```python
from build123d import *

# Parameters (mm, degrees)
SPANNER_BODY_3MM_DEPTH          = 3
HEAD_PAD_13_SIDE_A_DEPTH        = 1
HEAD_START                      = 1
HEAD_PAD_13_SIDE_B_DEPTH        = 1
HEAD_PAD_9_SIDE_A_DEPTH         = 1
HEAD_PAD_9_SIDE_B_DEPTH         = 1
HANDLE_SLOT_SIDE_A_55X6_5_DEPTH = 0.7
HANDLE_SLOT_SIDE_B_55X6_5_DEPTH = 0.7


with BuildPart() as part:
    # Spanner Profile Sketch → Spanner Body 3mm (new body)
    with BuildSketch(Plane.XY):
        with BuildLine():
            ThreePointArc((0.335793671, 9.351551373), (4.669621374, 5.426922629), (6.845232579, 0))
            Line((6.845232579, 0), (107.225035612, 0))
            ThreePointArc((107.225035612, 0), (107.061451957, 3.049932803), (107.927329677, 5.978943813))
            Line((107.927329677, 5.978943813), (120.095812241, 10.407909262))
            ThreePointArc((120.095812241, 10.407909262), (111.608728128, 14.410482081), (102.447920261, 12.37804878))
            ThreePointArc((102.447920261, 12.37804878), (90.682307093, 7.25217294), (77.968765244, 5.5))
            Line((77.968765244, 5.5), (34.824560299, 5.5))
            ThreePointArc((34.824560299, 5.5), (21.256828973, 7.500925935), (8.844332774, 13.333333333))
            ThreePointArc((8.844332774, 13.333333333), (-5.944434547, 14.854753378), (-15.600963823, 3.551046014))
            Line((-15.600963823, 3.551046014), (0.335793671, 9.351551373))
        make_face()
        with BuildLine():
            Line((107.225035612, 0), (6.845232579, 0))
            ThreePointArc((6.845232579, 0), (6.928993977, -3.356876833), (6.150136107, -6.623223181))
            Line((6.150136107, -6.623223181), (-9.990209349, -12.497828498))
            ThreePointArc((-9.990209349, -12.497828498), (0.615850097, -15.988143377), (10.921993446, -11.692307692))
            ThreePointArc((10.921993446, -11.692307692), (18.183666088, -7.104008283), (26.622359024, -5.5))
            Line((26.622359024, -5.5), (85.627884786, -5.5))
            ThreePointArc((85.627884786, -5.5), (93.595318501, -6.924087505), (100.576115451, -11.02))
            ThreePointArc((100.576115451, -11.02), (115.204003038, -13.533970311), (124.379255248, -1.867356026))
            Line((124.379255248, -1.867356026), (112.37359154, -6.237060258))
            ThreePointArc((112.37359154, -6.237060258), (109.059269326, -3.729420365), (107.225035612, 0))
        make_face()
    extrude(amount=SPANNER_BODY_3MM_DEPTH)

    # Head Pad 13 Side A Sketch → Head Pad 13 Side A (add)
    with BuildSketch(Plane.XY.offset(3)):
        with BuildLine():
            Line((-15.600963823, 3.551046014), (0.335793671, 9.351551373))
            ThreePointArc((0.335793671, 9.351551373), (6.21600407, 2.446261863), (6.150136107, -6.623223181))
            Line((6.150136107, -6.623223181), (-9.990209349, -12.497828498))
            ThreePointArc((-9.990209349, -12.497828498), (15.10359657, 5.280281303), (-15.600963823, 3.551046014))
        make_face()
    extrude(amount=HEAD_PAD_13_SIDE_A_DEPTH)

    # Head Pad 13 Side B Sketch → Head Pad 13 Side B (add)
    with BuildSketch(Plane(origin=(0, 0, 0), x_dir=(-1, 0, 0), z_dir=(0, 0, -1)).offset(HEAD_START)):
        with BuildLine():
            Line((-0.335793671, 9.351551373), (15.600963823, 3.551046014))
            ThreePointArc((15.600963823, 3.551046014), (-15.10359657, 5.280281303), (9.990209349, -12.497828498))
            Line((9.990209349, -12.497828498), (-6.150136107, -6.623223181))
            ThreePointArc((-6.150136107, -6.623223181), (-6.21600407, 2.446261863), (-0.335793671, 9.351551373))
        make_face()
    extrude(amount=-HEAD_PAD_13_SIDE_B_DEPTH)

    # Head Pad 9 Side A Sketch → Head Pad 9 Side A (add)
    with BuildSketch(Plane(origin=(0, 0, 0), x_dir=(-1, 0, 0), z_dir=(0, 0, -1)).offset(HEAD_START)):
        with BuildLine():
            Line((-107.927329677, 5.978943813), (-120.095812241, 10.407909262))
            ThreePointArc((-120.095812241, 10.407909262), (-96.309573907, -4.777262123), (-124.379255248, -1.867356026))
            Line((-124.379255248, -1.867356026), (-112.37359154, -6.237060258))
            ThreePointArc((-112.37359154, -6.237060258), (-107.542766412, -1.07818129), (-107.927329677, 5.978943813))
        make_face()
    extrude(amount=-HEAD_PAD_9_SIDE_A_DEPTH)

    # Head Pad 9 Side B Sketch → Head Pad 9 Side B (add)
    with BuildSketch(Plane.XY.offset(3)):
        with BuildLine():
            Line((107.927329677, 5.978943813), (120.095812241, 10.407909262))
            ThreePointArc((120.095812241, 10.407909262), (96.309573907, -4.777262123), (124.379255248, -1.867356026))
            Line((124.379255248, -1.867356026), (112.37359154, -6.237060258))
            ThreePointArc((112.37359154, -6.237060258), (107.542766412, -1.07818129), (107.927329677, 5.978943813))
        make_face()
    extrude(amount=HEAD_PAD_9_SIDE_B_DEPTH)

    # Handle Slot Side A Sketch → Handle Slot Side A 55x6.5 (cut)
    with BuildSketch(Plane.XY.offset(3)):
        with BuildLine():
            Line((28.768116085, 3.25), (83.753668591, 3.25))
            ThreePointArc((83.753668591, 3.25), (87.003668591, 0), (83.753668591, -3.25))
            Line((83.753668591, -3.25), (28.753668591, -3.250032112))
            ThreePointArc((28.753668591, -3.250032112), (25.503644507, 0.007223765), (28.768116085, 3.25))
        make_face()
    extrude(amount=-HANDLE_SLOT_SIDE_A_55X6_5_DEPTH, mode=Mode.SUBTRACT)

    # Handle Slot Side B Sketch → Handle Slot Side B 55x6.5 (cut)
    with BuildSketch(Plane(origin=(0, 0, 0), x_dir=(-1, 0, 0), z_dir=(0, 0, -1))):
        with BuildLine():
            Line((-83.625121905, 3.25), (-28.625121905, 3.25))
            ThreePointArc((-28.625121905, 3.25), (-25.375121905, 0), (-28.625121905, -3.25))
            Line((-28.625121905, -3.25), (-83.625121905, -3.25))
            ThreePointArc((-83.625121905, -3.25), (-86.875121905, 0), (-83.625121905, 3.25))
        make_face()
    extrude(amount=-HANDLE_SLOT_SIDE_B_55X6_5_DEPTH, mode=Mode.SUBTRACT)


solid = part.part
```
Model file for the job. Use its own axes, mm. A direction names the side the tool comes from. Coordinates: 2 decimals unless noted, no trailing zeros. Order: outer loops, then holes, each group sorted by start corner. A loop starts at its lowest first (then second) coordinate and runs counter-clockwise, first axis right, second up. Notation, with made-up numbers: (75, -29.5) - (131, -29.5) arc R15 cw to (131, -6.5) - close; hole circle Ø2 at (-29, 86.25). An arc over 180 degrees is marked (long way). Return JSON: item names as keys, results as strings. Group by question number.
1) Saw through at D-D, the plane x = 94. Write the cut outline in (y, z).
2) Tool access for faces 4 (the flat face through (-2.03, -9.6, 1.46)), 5 (the cylindrical face through (86.874, -0.071, 0.345)), 6 (the flat face through (113.926, 8.162, 1.465)), 7 (the cylindrical face through (90.856, 7.301, 1.479)), 8 (the flat face through (57, 0, 2.3)): list every direction of +Z, -Z, +X, -X, +Y, -Y with a clear straight run to the whole face (end or side of a thin tool).
3) Flat gauge pins, fed straight in: P1, Ø5, axis at x = 51.5, y = 0, coming from the +Z side; P2, Ø2.5, axis at x = 54, z = 2, coming from the -Y side; P3, Ø0.9, axis at x = 58.5, z = 1, coming from the +Y side. Where does each tip first touch, or does it go through?
4) Saw through at C-C, the plane y = -9.5. Write the cut outline in (x, z), plus the area to 3 significant figures.
5) Probe line 1 (Y direction, x = 66.5, z = 2.9); line 2 (X direction, y = 11, z = 0.05). List the from-to ranges inside material, lowest first. Write a range as from..to.
6) Saw through at A-A, the plane x = 114.5. Write the cut outline in (y, z), plus the area to 3 significant figures.
7) Saw through at B-B, the plane x = 41.5. Write the cut outline in (y, z).
8) Mould opens along Y. For faces 1 (the cylindrical face through (93.488, -6.885, 1.479)), 2 (the flat face through (55, 5, 3)), 3 (the cylindrical face through (87.003, 0.071, 2.655)) say: released by +Y, released by -Y, zero draft, split by the parting line, or undercut.
Values found:
{
 "1": {"outline": "(-7.08, 0) - (8.32, 0) - (8.32, 3) - (-7.08, 3) - close"},
 "2": {"face 4": "+Z, -Z, -X", "face 5": "-Z", "face 6": "+Z, -Z, +X", "face 7": "+Z, -Z, +Y", "face 8": "+Z"},
 "3": {"P1": "stops at z = 2.3", "P2": "stops at y = -5.5", "P3": "stops at y = 5.5"},
 "4": {"outline": "(-1.75, -1) - (12.87, -1) - (12.87, 0) - (13.66, 0) - (13.66, 3) - (12.87, 3) - (12.87, 4) - (-1.75, 4) - close; (98.59, 0) - (99.05, 0) - (99.05, -1) - (120.95, -1) - (120.95, 4) - (99.05, 4) - (99.05, 3) - (98.59, 3) - close", "area": "186 mm²"},
 "5": {"line 1": "y = -5.5..-3.25, 3.25..5.5", "line 2": "x = -11.62..12.76, 100.03..119.45"},
 "6": {"outline": "(-13.78, -1) - (-5.46, -1) - (-5.46, 4) - (-13.78, 4) - close; (8.37, -1) - (13.78, -1) - (13.78, 4) - (8.37, 4) - close", "area": "68.7 mm²"},
 "7": {"outline": "(-5.5, 0) - (-3.25, 0) - (-3.25, 0.7) - (3.25, 0.7) - (3.25, 0) - (5.5, 0) - (5.5, 3) - (3.25, 3) - (3.25, 2.3) - (-3.25, 2.3) - (-3.25, 3) - (-5.5, 3) - close"},
 "8": {"face 1": "released by -Y", "face 2": "zero draft", "face 3": "undercut"}
}
